```python
from build123d import *

# Parameters (mm, degrees)
SKETCH1_R                               = 31
SKETCH1_R_2                             = 20
BOSS_EXTRUDE1_DEPTH                     = 67
SKETCH2_W                               = 75
SKETCH2_H                               = 75
SKETCH2_R                               = 20
BOSS_EXTRUDE2_DEPTH                     = 13
CBORE_FOR_M8_HEX_HEAD_BOLT1_D           = 9
CBORE_FOR_M8_HEX_HEAD_BOLT1_CBORE_D     = 18
CBORE_FOR_M8_HEX_HEAD_BOLT1_CBORE_DEPTH = 8
CHAMFER1_SIZE                           = 2


with BuildPart() as part:
    # Sketch1 → Boss-Extrude1 (new body)
    with BuildSketch(Plane(origin=(0, 0, 0), x_dir=(0, 0, -1), z_dir=(1, 0, 0))):
        Circle(SKETCH1_R)
        Circle(SKETCH1_R_2, mode=Mode.SUBTRACT)
    extrude(amount=BOSS_EXTRUDE1_DEPTH)

    # Sketch2 → Boss-Extrude2 (add)
    with BuildSketch(Plane(origin=(67, 0, 0), x_dir=(0, 0, -1), z_dir=(1, 0, 0))):
        Rectangle(SKETCH2_W, SKETCH2_H)
        Circle(SKETCH2_R, mode=Mode.SUBTRACT)
    extrude(amount=BOSS_EXTRUDE2_DEPTH)

    # CBORE for M8 Hex Head Bolt1 (through all)
    with Locations(Plane(origin=(80, 0, 0), x_dir=(0, 0, -1), z_dir=(1, 0, 0))):
        with Locations((28.284271247, 28.284271247), (28.284271247, -28.284271247), (-28.284271247, -28.284271247), (-28.284271247, 28.284271247)):
            CounterBoreHole(CBORE_FOR_M8_HEX_HEAD_BOLT1_D / 2, CBORE_FOR_M8_HEX_HEAD_BOLT1_CBORE_D / 2, CBORE_FOR_M8_HEX_HEAD_BOLT1_CBORE_DEPTH)

    # Chamfer1
    chamfer1_edges = [part.edges().sort_by_distance(p)[0] for p in [
        (73.5, -37.5, -37.5),
        (73.5, 37.5, -37.5),
        (73.5, 37.5, 37.5),
        (73.5, -37.5, 37.5),
    ]]
    chamfer(chamfer1_edges, length=CHAMFER1_SIZE)


solid = part.part
```
Geometry check sheet. Reference: the model listing, model coordinates, mm. A direction names the side the tool comes from. Coordinates: 2 decimals unless noted, no trailing zeros. Write each loop counter-clockwise with the first axis right and the second up, starting at its lowest first coordinate (ties: lowest second). Pieces come first, ordered by that corner, then holes. Notation, with made-up numbers: M 82,37 L 129,37 A23 ccw 129,61 Z; hole C 7.5,66.5 d11. An arc over 180 degrees is marked long. One line per item, written item: value. Start each with the question number.
(1) Sectioned sample at D-D, the plane z = 26. Enter the section's corners in (x, y), and give its area (3 significant figures).
(2) Scan lines: line 1 along Y through (x, z) = (28, 0); line 2 along X through (y, z) = (-22.5, 28.5); line 3 along Z through (x, y) = (32.5, -14.5). Record each from-to range of solid material in increasing order. Write a range as [from, to].
(3) Sectioned sample at A-A, the plane z = 0. Enter the section's corners in (x, y).
(4) Depth check by flat-ended pin: pin 1 (8 mm diameter, centred on y = -28.28, z = 28.28, fed in from +X); pin 2 (5.5 mm diameter, centred on y = -25.5, z = -27, fed in from +X); pin 3 (2 mm diameter, centred on x = 46, y = -23.5, fed in from -Z); pin 4 (10.5 mm diameter, centred on y = 28.28, z = -28.28, fed in from -X). Enter the tip coordinate at first touch or a pass-through.
(5) Release check for a two-part mould opening along Y. For faces 4 (the face through (72, -24, 26)), 5 (the face through (80, -16, -16)), 6 (the face through (73, -37, 36)) record: released by +Y, released by -Y, zero draft, split by the parting line, or undercut.
(6) Sectioned sample at C-C, the plane x = 74. Enter the section's corners in (y, z).
(7) Tool access check on faces 1 (the face through (69.46, 24.29, -26.21)), 2 (the face through (67, 1, -33)), 3 (the face through (72, -24, -26)). Record the directions out of +Z, -Z, +X, -X, +Y, -Y that give a thin tool (end or side, any length) a straight path to the whole face; none if there is none.
Filled sheet:
1. outline: M 0,-16.88 L 67,-16.88 L 67,-24.41 L 72,-24.41 L 72,-19.58 L 80,-19.58 L 80,19.58 L 72,19.58 L 72,24.41 L 67,24.41 L 67,16.88 L 0,16.88 Z; M 67,-37.5 L 80,-37.5 L 80,-36.99 L 72,-36.99 L 72,-32.16 L 67,-32.16 Z; M 67,32.16 L 72,32.16 L 72,36.99 L 80,36.99 L 80,37.5 L 67,37.5 Z
1. area: 2,880 mm²
2. line 1: [-31, -20], [20, 31]
2. line 2: [67, 72]
2. line 3: [-27.4, -13.77], [13.77, 27.4]
3. outline: M 0,-31 L 67,-31 L 67,-37.5 L 80,-37.5 L 80,-20 L 0,-20 Z; M 0,20 L 80,20 L 80,37.5 L 67,37.5 L 67,31 L 0,31 Z
4. pin 1: through
4. pin 2: x = 72
4. pin 3: z = -21.32
4. pin 4: x = 67
5. face 4: undercut
5. face 5: zero draft
5. face 6: released by -Y
6. outline: M -37.5,-35.5 L -35.5,-37.5 L 35.5,-37.5 L 37.5,-35.5 L 37.5,35.5 L 35.5,37.5 L -35.5,37.5 L -37.5,35.5 Z; hole C -28.28,-28.28 d18; hole C -28.28,28.28 d18; hole C 0,0 d40; hole C 28.28,-28.28 d18; hole C 28.28,28.28 d18
7. face 1: +X, -X
7. face 2: -X
7. face 3: +X
